```python
from build123d import *

# Parameters (mm, degrees)
EXTRUDE_1_DEPTH     = 1.5
SKETCH_4_R          = 2.5
CUT_EXTRUDE_1_DEPTH = 1.5
SKETCH_5_R          = 30
EXTRUDE_2_DEPTH     = 15
SKETCH_10_R         = 4
EXTRUDE_3_DEPTH     = 10


with BuildPart() as part:
    # 草图1 → 凸台-拉伸1 (new body)
    with BuildSketch(Plane.XY):
        with BuildLine():
            ThreePointArc((-28.118568833, 48.655761142), (-14.710337472, 42.212909992), (0, 40))
            ThreePointArc((0, 40), (18.246546062, 43.448270099), (33.976331356, 53.317457727))
            Line((33.976331356, 53.317457727), (59.220103302, 72.989737675))
            ThreePointArc((59.220103302, 72.989737675), (72.664625967, 70.256318884), (70.727374666, 56.674204713))
            Line((70.727374666, 56.674204713), (48.655761142, 28.118568833))
            ThreePointArc((48.655761142, 28.118568833), (42.212909992, 14.710337472), (40, 0))
            ThreePointArc((40, 0), (43.448270099, -18.246546062), (53.317457727, -33.976331356))
            Line((53.317457727, -33.976331356), (72.989737675, -59.220103302))
            ThreePointArc((72.989737675, -59.220103302), (70.256318884, -72.664625967), (56.674204713, -70.727374666))
            Line((56.674204713, -70.727374666), (28.118568833, -48.655761142))
            ThreePointArc((28.118568833, -48.655761142), (14.710337472, -42.212909992), (0, -40))
            ThreePointArc((0, -40), (-18.246546062, -43.448270099), (-33.976331356, -53.317457727))
            Line((-33.976331356, -53.317457727), (-59.220103302, -72.989737675))
            ThreePointArc((-59.220103302, -72.989737675), (-72.664625967, -70.256318884), (-70.727374666, -56.674204713))
            Line((-70.727374666, -56.674204713), (-48.655761142, -28.118568833))
            ThreePointArc((-48.655761142, -28.118568833), (-42.212909992, -14.710337472), (-40, 0))
            ThreePointArc((-40, 0), (-43.448270099, 18.246546062), (-53.317457727, 33.976331356))
            Line((-53.317457727, 33.976331356), (-72.989737675, 59.220103302))
            ThreePointArc((-72.989737675, 59.220103302), (-70.256318884, 72.664625967), (-56.674204713, 70.727374666))
            Line((-56.674204713, 70.727374666), (-28.118568833, 48.655761142))
        make_face()
    extrude(amount=EXTRUDE_1_DEPTH)

    # 草图4 → 切除-拉伸1 (cut)
    with BuildSketch(Plane.XY.offset(1.5)):
        with Locations((-50, 50)):
            Circle(SKETCH_4_R)
        with Locations((-37.5, 37.5)):
            Circle(SKETCH_4_R)
        with Locations((50, 50)):
            Circle(SKETCH_4_R)
        with Locations((37.5, 37.5)):
            Circle(SKETCH_4_R)
        with Locations((50, -50)):
            Circle(SKETCH_4_R)
        with Locations((37.5, -37.5)):
            Circle(SKETCH_4_R)
        with Locations((-50, -50)):
            Circle(SKETCH_4_R)
        with Locations((-37.5, -37.5)):
            Circle(SKETCH_4_R)
    extrude(amount=-CUT_EXTRUDE_1_DEPTH, mode=Mode.SUBTRACT)

    # 草图5 → 凸台-拉伸2 (add)
    with BuildSketch(Plane.XY.offset(1.5)):
        Circle(SKETCH_5_R)
    extrude(amount=EXTRUDE_2_DEPTH)

    # 草图6 → 切除-旋转1 (revolve, cut)
    with BuildSketch(Plane(origin=(0, 0, 0), x_dir=(1, 0, 0), z_dir=(0, 1, 0)), mode=Mode.PRIVATE) as cut_revolve_1_sk:
        with BuildLine():
            Line((30, -16.5), (30, -6.799483709))
            add(Edge.make_bspline(
                [(30, -6.799483709), (23.649728085, -14.104545992), (14.118358568, -16.5)],
                knots=[0, 0, 0, 1, 1, 1], degree=2))
            Line((14.118358568, -16.5), (30, -16.5))
        make_face()
    revolve(cut_revolve_1_sk.sketch.rotate(Axis((0, 0, 0), (0, 0, 1)), 180), axis=Axis((0, 0, 0), (0, 0, 1)), mode=Mode.SUBTRACT)

    # 草图10 → 凸台-拉伸3 (add)
    with BuildSketch(Plane.XY.offset(16.5)):
        Circle(SKETCH_10_R)
    extrude(amount=EXTRUDE_3_DEPTH)


solid = part.part
```
Could you check a few things on this model? Use its own coordinates, in mm. A direction names the side the tool comes from. Give positions to 0.01 mm unless a question says otherwise; leave off trailing zeros. Write each loop counter-clockwise with the first axis right and the second up, starting at its lowest first coordinate (ties: lowest second). Pieces come first, ordered by that corner, then holes. Notation, with made-up numbers: (-37, -5.75) - (-12, -5.75) arc R31 ccw to (-12, 20.25) - close; hole circle Ø7 at (80, 88.25). An arc over 180 degrees is marked (long way). One line per item, written item: value. Start each with the question number.
Item 1: Which directions (+Z, -Z, +X, -X, +Y, -Y) give clear straight access to the entire face, cutting with the end or side of a thin tool? Please do faces 1 (the face through (-35.19, 36.54, 0.76)), 2 (the face through (46.4, 63, 0.7)), 3 (the face through (-59.85, -42.6, 0.74)), 4 (the face through (1, 1, 0)), 5 (the face through (-0.867, -3.905, 21.43)).
Item 2: Imagine slicing it at C-C, the plane y = -65. List the corners of the cut face in (x, z) for me.
Item 3: I'm going to push flat-ended pins straight in: pin 1 (6 mm diameter, centred on x = -37.5, y = 37.5, fed in from +Z); pin 2 (8 mm diameter, centred on y = -0.5, z = 23.5, fed in from -X); pin 3 (1 mm diameter, centred on x = 42, y = 56.5, fed in from -Z). Where does each tip first touch, or does it pass through?
Item 4: Imagine slicing it at B-B, the plane y = 44. List the corners of the cut face in (x, z) for me.
Item 5: Imagine slicing it at A-A, the plane x = -37. List the corners of the cut face in (y, z) for me.
Item 6: If we mould it in two halves opening along Y, with no side actions, what happens to faces 6 (the face through (72.54, 70.43, 0.74)), 7 (the face through (42.6, -59.85, 0.74)), 8 (the face through (-32, 1, 1.5)), 9 (the face through (59.85, 42.6, 0.74))? For each: +Y half, -Y half, draft (parallel to the pull), parting line (faces both ways), or undercut.
Item 7: Please list where these lines run through material, in increasing order: line 1 (Y direction, x = 37.5, z = 1.1); line 2 (Y direction, x = 50, z = 0.85); line 3 (Z direction, x = -34, y = 32). Write a range as from..to.
Geometry says:
1. face 1: +Z, -Z
1. face 2: +Z, -Z, +Y
1. face 3: +Z, -Z, -X
1. face 4: -Z, +X, -X, +Y, -Y
1. face 5: +Z
2. outline: (-74.48, 0) - (-48.97, 0) - (-48.97, 1.5) - (-74.48, 1.5) - close; (49.26, 0) - (74.48, 0) - (74.48, 1.5) - (49.26, 1.5) - close
3. pin 1: z = 1.5
3. pin 2: x = -4
3. pin 3: z = 0
4. outline: (-61.13, 0) - (-19.6, 0) - (-19.6, 1.5) - (-61.13, 1.5) - close; (19.6, 0) - (60.93, 0) - (60.93, 1.5) - (19.6, 1.5) - close
5. outline: (-55.67, 0) - (-39.95, 0) - (-39.95, 1.5) - (-55.67, 1.5) - close; (-35.05, 0) - (35.05, 0) - (35.05, 1.5) - (-35.05, 1.5) - close; (39.95, 0) - (55.52, 0) - (55.52, 1.5) - (39.95, 1.5) - close
6. face 6: undercut
6. face 7: -Y half
6. face 8: draft
6. face 9: undercut
7. line 1: -55.91..-40, -35..35, 40..56.06
7. line 2: -65.57..-52.5, -47.5..-30, 29.86..47.5, 52.5..65.8
7. line 3: 0..1.5
